CAD build for the part. Positions are in the model's coordinates, mm. Face numbers are marked on the shaded views. A direction names the side the tool comes from. Coordinates: 2 decimals unless noted, no trailing zeros. Order: outer loops, then holes, each group sorted by start corner. A loop starts at its lowest first (then second) coordinate and runs counter-clockwise, first axis right, second up. Notation, with made-up numbers: (-3.5, -29.5) - (43.5, -29.5) arc R27 ccw to (43.5, -7.5) - close; hole circle Ø6 at (31.25, 49.25). An arc over 180 degrees is marked (long way). Return JSON: item names as keys, results as strings.
from build123d import *

# Parameters (mm, degrees)
BOSS_EXTRUDE1_DEPTH = 10
SKETCH2_R           = 4
BOSS_EXTRUDE2_DEPTH = 125
BOSS_EXTRUDE3_START = 125
SKETCH3_R           = 4
BOSS_EXTRUDE3_DEPTH = 125


with BuildPart() as part:
    # Sketch1 → Boss-Extrude1 (new body)
    with BuildSketch(Plane.XY):
        with BuildLine():
            Line((-4.5, 71), (4.5, 71))
            ThreePointArc((4.5, 71), (10.156854249, 68.656854249), (12.5, 63))
            Line((12.5, 63), (12.5, -63))
            ThreePointArc((12.5, -63), (10.156854249, -68.656854249), (4.5, -71))
            Line((4.5, -71), (-4.5, -71))
            ThreePointArc((-4.5, -71), (-10.156854249, -68.656854249), (-12.5, -63))
            Line((-12.5, -63), (-12.5, 63))
            ThreePointArc((-12.5, 63), (-10.156854249, 68.656854249), (-4.5, 71))
        make_face()
        with BuildLine():
            Line((-4.5, 66), (4.5, 66))
            ThreePointArc((4.5, 66), (6.621320344, 65.121320344), (7.5, 63))
            Line((7.5, 63), (7.5, -63))
            ThreePointArc((7.5, -63), (6.621320344, -65.121320344), (4.5, -66))
            Line((4.5, -66), (-4.5, -66))
            ThreePointArc((-4.5, -66), (-6.621320344, -65.121320344), (-7.5, -63))
            Line((-7.5, -63), (-7.5, 63))
            ThreePointArc((-7.5, 63), (-6.621320344, 65.121320344), (-4.5, 66))
        make_face(mode=Mode.SUBTRACT)
    extrude(amount=BOSS_EXTRUDE1_DEPTH)

    # Sketch2 → Boss-Extrude2 (add)
    with BuildSketch(Plane(origin=(12.5, 0, 0), x_dir=(0, 0, -1), z_dir=(1, 0, 0))):
        with Locations(Location((-5, 0, 0), (0, 0, 270))):
            Circle(SKETCH2_R)
    extrude(amount=BOSS_EXTRUDE2_DEPTH)

    # Sketch3 → Boss-Extrude3 (add)
    with BuildSketch(Plane.ZY.offset(12.5).offset(BOSS_EXTRUDE3_START)):
        with Locations(Location((5, 0, 0), (0, 0, 270))):
            Circle(SKETCH3_R)
    extrude(amount=-BOSS_EXTRUDE3_DEPTH)


solid = part.part
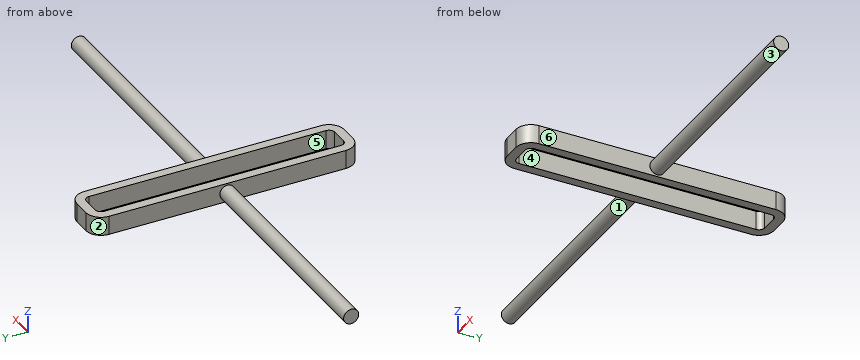
Item 1: Mould opens along X. For the marked faces 3, 4, 5 and 6 say: released by +X, released by -X, zero draft, split by the parting line, or undercut.
Findings below:
{"face 3": "zero draft", "face 4": "undercut", "face 5": "undercut", "face 6": "released by +X"}
Item 2: Which spindle directions (+Z, -Z, +X, -X, +Y, -Y) get a long thin tool onto all of the face, cutting with end or side? Do the marked faces 1 and 2. Say none if no direction does.
Findings below:
{"face 1": "-X", "face 2": "+Z, -Z, -X, +Y"}
Item 3: Wall check: L1, parallel to X at y = -10.5, z = 4.5; L2, parallel to X at y = -1.5, z = 7; L3, parallel to Y at x = 102, z = 7.5. Give the ranges that are in metal, low to high. Write a range as [from, to].
Findings below:
{"L1": "x = [-12.5, -7.5], [7.5, 12.5]", "L2": "x = [-137.5, -7.5], [7.5, 137.5]", "L3": "y = [-3.12, 3.12]"}
Item 4: Drop flat-ended pins along their axis: P1, Ø2, axis at y = 48, z = 4, coming from the +X side; P2, Ø5, axis at y = -15.5, z = 4, coming from the -X side; P3, Ø1.5, axis at x = 71.5, z = 6.5, coming from the -Y side. Give the stop position or say it passes through.
Findings below:
{"P1": "stops at x = 12.5", "P2": "stops at x = -12.5", "P3": "stops at y = -3.93"}
Item 5: Band-saw the part on A-A, the plane y = 0. List the corners of the cut face in (x, z).
Findings below:
{"outline": "(-137.5, 1) - (-12.5, 1) - (-12.5, 0) - (-7.5, 0) - (-7.5, 10) - (-12.5, 10) - (-12.5, 9) - (-137.5, 9) - close; (7.5, 0) - (12.5, 0) - (12.5, 1) - (137.5, 1) - (137.5, 9) - (12.5, 9) - (12.5, 10) - (7.5, 10) - close"}
Item 6: Band-saw the part on C-C, the plane x = 118.5. List the corners of the cut face in (y, z).
Findings below:
{"outline": "circle Ø8 at (0, 5)"}
Item 7: Band-saw the part on B-B, the plane z = 5. List the corners of the cut face in (x, y), then the cut area to 3 significant figures.
Findings below:
{"outline": "(-137.5, -4) - (-12.5, -4) - (-12.5, -63) arc R8 ccw to (-4.5, -71) - (4.5, -71) arc R8 ccw to (12.5, -63) - (12.5, -4) - (137.5, -4) - (137.5, 4) - (12.5, 4) - (12.5, 63) arc R8 ccw to (4.5, 71) - (-4.5, 71) arc R8 ccw to (-12.5, 63) - (-12.5, 4) - (-137.5, 4) - close; hole (-7.5, -63) arc R3 ccw to (-4.5, -66) - (4.5, -66) arc R3 ccw to (7.5, -63) - (7.5, 63) arc R3 ccw to (4.5, 66) - (-4.5, 66) arc R3 ccw to (-7.5, 63) - close", "area": "3,520 mm²"}
